Design review of the part built by this model. Coordinates are the model's own, in mm. A direction names the side the tool comes from. Coordinates: 2 decimals unless noted, no trailing zeros. Write each loop counter-clockwise with the first axis right and the second up, starting at its lowest first coordinate (ties: lowest second). Pieces come first, ordered by that corner, then holes. Notation, with made-up numbers: (32, 11.5) -> (59, 11.5) arc R25 cw to (59, 30.5) -> close; hole circle Ø6 at (-19, 67). An arc over 180 degrees is marked (long way). Answer in a Markdown table with one row per item. Add a question column.
Item 1: Clearance check with flat-ended pins moving along their axes: P1, Ø1.8, axis at x = 0, y = -17, coming from the +Z side; P2, Ø1, axis at y = -6.5, z = -1, coming from the +X side; P3, Ø3, axis at x = 3, z = -2.5, coming from the +Y side. State where each tip first meets the part, or that it passes through.
Item 2: Take a section at D-D, the plane y = -16.25. Write out the cut boundary in (x, z) (3 decimals), and give its area (3 significant figures).
Item 3: Take a section at A-A, the plane x = 0. Write out the cut boundary in (y, z).
Item 4: For faces 1 (the face through (-0.867, -1.26, 3.905)), 2 (the face through (-3, -2, -1)), list the 3-axis set-ups (+Z, -Z, +X, -X, +Y, -Y) from which the entire face can be reached by the end or side of a thin tool; tool diameter is ignored.
Item 5: Take a section at B-B, the plane z = 0. Write out the cut boundary in (x, y), and give its area (3 significant figures).
Item 6: To check wall thickness, follow line 1 (Y direction, x = 0, z = -0.1); line 2 (X direction, y = -17, z = 0.15); line 3 (Y direction, x = 0.5, z = -1.75). State the ranges of each line that lie inside material, in increasing order.
Item 7: Draft analysis for pull direction X (two halves, no side actions). For faces 3 (the face through (0, -20, 0)), 4 (the face through (0, -18, 0)), 5 (the face through (2.17, -11.12, 0.9)), state which applies: released by +X, released by -X, zero draft, split by the parting line, or undercut.
Item 8: Take a section at C-C, the plane y = -5.75. Write out the cut boundary in (x, z).
from build123d import *

# Parameters (mm, degrees)
FILLET1_R               = 0.5
CHAMFER1_SIZE           = 0.5
CUT_EXTRUDE1_DEPTH      = 21.784609691
CUT_EXTRUDE1_DEPTH_BACK = 21.784609691
SKETCH2_R               = 1


with BuildPart() as part:
    # Sketch1 → Revolve1 (revolve)
    with BuildSketch(Plane.XY):
        Polygon((0, 0), (4, 0), (4, -2), (2.35, -2), (2.35, -20), (0, -20), align=None)
    revolve(axis=Axis((0, -273.133875929, 0), (0, 1, 0)))

    # Fillet1
    fillet1_edges = [part.edges().sort_by_distance(p)[0] for p in [
        (-2.35, -2, 0),
    ]]
    fillet(fillet1_edges, radius=FILLET1_R)

    # Chamfer1
    chamfer1_edges = [part.edges().sort_by_distance(p)[0] for p in [
        (-2.35, -20, 0),
        (-4, 0, 0),
    ]]
    chamfer(chamfer1_edges, length=CHAMFER1_SIZE)

    # Sketch2 → Cut-Extrude1 (cut, two sides: drawn at the far end of the back side and taken through both)
    with BuildSketch(Plane.XY.offset(-CUT_EXTRUDE1_DEPTH_BACK)):
        with Locations((0, -17)):
            Circle(SKETCH2_R)
    extrude(amount=CUT_EXTRUDE1_DEPTH + CUT_EXTRUDE1_DEPTH_BACK, mode=Mode.SUBTRACT)


solid = part.part
Answers:
| question | item | result |
|---|---|---|
| 1 | P1 | passes through |
| 1 | P2 | stops at x = 2.3 |
| 1 | P3 | stops at y = 0 |
| 2 | outline | (-0.661, -2.255) -> (-0.661, 2.255) arc R2.35 ccw to start; (0.661, -2.255) arc R2.35 ccw to (0.661, 2.255) -> close |
| 2 | area | 11.2 mm^2 |
| 3 | outline | (-20, -1.85) -> (-19.5, -2.35) -> (-18, -2.35) -> (-18, 2.35) -> (-19.5, 2.35) -> (-20, 1.85) -> close; (-16, -2.35) -> (-2.5, -2.35) arc R0.5 cw to (-2, -2.85) -> (-2, -4) -> (-0.5, -4) -> (0, -3.5) -> (0, 3.5) -> (-0.5, 4) -> (-2, 4) -> (-2, 2.85) arc R0.5 cw to (-2.5, 2.35) -> (-16, 2.35) -> close |
| 4 | face 1 | +Y, -Y |
| 4 | face 2 | -Y |
| 5 | outline | (-4, -2) -> (-2.85, -2) arc R0.5 cw to (-2.35, -2.5) -> (-2.35, -19.5) -> (-1.85, -20) -> (1.85, -20) -> (2.35, -19.5) -> (2.35, -2.5) arc R0.5 cw to (2.85, -2) -> (4, -2) -> (4, -0.5) -> (3.5, 0) -> (-3.5, 0) -> (-4, -0.5) -> close; hole circle Ø2 at (0, -17) |
| 5 | area | 97.1 mm^2 |
| 6 | line 1 | y = -20 to -18, -16 to 0 |
| 6 | line 2 | x = -2.35 to -1, 1 to 2.35 |
| 6 | line 3 | y = -20 to -17.87, -16.13 to 0 |
| 7 | face 3 | zero draft |
| 7 | face 4 | undercut |
| 7 | face 5 | split by the parting line |
| 8 | outline | circle Ø4.7 at (0, 0) |
